```python
from build123d import *

# Parameters (mm, degrees)
SKETCH1_W                                        = 435
SKETCH1_H                                        = 385
BOSS_EXTRUDE1_DEPTH                              = 4
FILLET1_R                                        = 20
SKETCH2_R                                        = 1.555451355
SKETCH2_R_2                                      = 1.5
SKETCH2_R_3                                      = 1.924870622
CUT_EXTRUDE1_DEPTH                               = 10
CUT_EXTRUDE2_DEPTH                               = 4
HOLE_SIZE_BY_HEXALOBULAR_COUNTERSUNK_D           = 6.6
HOLE_SIZE_BY_HEXALOBULAR_COUNTERSUNK_DEPTH       = 7.5
HOLE_SIZE_BY_HEXALOBULAR_COUNTERSUNK_CSINK_D     = 12.8
HOLE_SIZE_BY_HEXALOBULAR_COUNTERSUNK_CSINK_ANGLE = 90
HOLE_SIZE_BY_HEXALOBULAR_COUNTERSUNK_TIP         = 1.982840043
SKETCH6_R                                        = 17.5
CUT_EXTRUDE3_DEPTH                               = 4
SKETCH7_R                                        = 1.6
CUT_EXTRUDE4_DEPTH                               = 4


with BuildPart() as part:
    # Sketch1 → Boss-Extrude1 (new body)
    with BuildSketch(Plane(origin=(0, 0, 0), x_dir=(1, 0, 0), z_dir=(0, 1, 0))):
        Rectangle(SKETCH1_W, SKETCH1_H)
    extrude(amount=BOSS_EXTRUDE1_DEPTH)

    # Fillet1
    fillet1_edges = [part.edges().sort_by_distance(p)[0] for p in [
        (217.5, 2, 192.5),
        (-217.5, 2, 192.5),
        (-217.5, 2, -192.5),
        (217.5, 2, -192.5),
    ]]
    fillet(fillet1_edges, radius=FILLET1_R)

    # Sketch2 → Cut-Extrude1 (cut)
    with BuildSketch(Plane(origin=(0, 4, 0), x_dir=(1, 0, 0), z_dir=(0, 1, 0))):
        with Locations(Location((-42.5, 0, 0), (0, 0, 270))):
            Circle(SKETCH2_R)
        with Locations(Location((-55.5, 7.5, 0), (0, 0, 270))):
            Circle(SKETCH2_R_2)
        with Locations(Location((-55.5, -7.5, 0), (0, 0, 270))):
            Circle(SKETCH2_R_3)
    extrude(amount=-CUT_EXTRUDE1_DEPTH, mode=Mode.SUBTRACT)

    # Sketch3 → Cut-Extrude2 (cut)
    with BuildSketch(Plane(origin=(0, 4, 0), x_dir=(1, 0, 0), z_dir=(0, 1, 0))):
        with BuildLine():
            Line((-24.5, -25), (69.5, -25))
            ThreePointArc((69.5, -25), (71.621320344, -24.121320344), (72.5, -22))
            Line((72.5, -22), (72.5, 22))
            ThreePointArc((72.5, 22), (71.621320344, 24.121320344), (69.5, 25))
            Line((69.5, 25), (-24.5, 25))
            ThreePointArc((-24.5, 25), (-26.621320344, 24.121320344), (-27.5, 22))
            Line((-27.5, 22), (-27.5, -22))
            ThreePointArc((-27.5, -22), (-26.621320344, -24.121320344), (-24.5, -25))
        make_face()
    extrude(amount=-CUT_EXTRUDE2_DEPTH, mode=Mode.SUBTRACT)

    # Hole Size (% by) Hexalobular Countersunk Head Screw Type1
    with Locations(Plane(origin=(0, 4, 0), x_dir=(1, 0, 0), z_dir=(0, 1, 0))):
        with Locations((-55.5, -7.5), (-42.5, 0), (-55.5, 7.5)):
            CounterSinkHole(HOLE_SIZE_BY_HEXALOBULAR_COUNTERSUNK_D / 2, HOLE_SIZE_BY_HEXALOBULAR_COUNTERSUNK_CSINK_D / 2, depth=HOLE_SIZE_BY_HEXALOBULAR_COUNTERSUNK_DEPTH, counter_sink_angle=HOLE_SIZE_BY_HEXALOBULAR_COUNTERSUNK_CSINK_ANGLE)
            with Locations((0, 0, -(HOLE_SIZE_BY_HEXALOBULAR_COUNTERSUNK_DEPTH + HOLE_SIZE_BY_HEXALOBULAR_COUNTERSUNK_TIP / 2))):  # 118° drill point
                Cone(0, HOLE_SIZE_BY_HEXALOBULAR_COUNTERSUNK_D / 2, HOLE_SIZE_BY_HEXALOBULAR_COUNTERSUNK_TIP, mode=Mode.SUBTRACT)

    # Sketch6 → Cut-Extrude3 (cut)
    with BuildSketch(Plane.XZ):
        with Locations(Location((-48, 100, 0), (0, 0, 270))):
            Circle(SKETCH6_R)
        with Locations(Location((97, 100, 0), (0, 0, 270))):
            Circle(SKETCH6_R)
        with Locations(Location((-48, -100, 0), (0, 0, 270))):
            Circle(SKETCH6_R)
        with Locations(Location((97, -100, 0), (0, 0, 270))):
            Circle(SKETCH6_R)
    extrude(amount=-CUT_EXTRUDE3_DEPTH, mode=Mode.SUBTRACT)

    # Sketch7 → Cut-Extrude4 (cut)
    with BuildSketch(Plane.XZ):
        with Locations(Location((-190, 175, 0), (0, 0, 270))):
            Circle(SKETCH7_R)
        with Locations(Location((-190, 0, 0), (0, 0, 270))):
            Circle(SKETCH7_R)
        with Locations(Location((-190, -175, 0), (0, 0, 270))):
            Circle(SKETCH7_R)
        with Locations(Location((190, 175, 0), (0, 0, 270))):
            Circle(SKETCH7_R)
        with Locations(Location((190, 0, 0), (0, 0, 270))):
            Circle(SKETCH7_R)
        with Locations(Location((190, -175, 0), (0, 0, 270))):
            Circle(SKETCH7_R)
    extrude(amount=-CUT_EXTRUDE4_DEPTH, mode=Mode.SUBTRACT)


solid = part.part
```
For this review, take the finished solid that the model builds, in its own axes (mm). Coordinates: 2 decimals unless noted, no trailing zeros. Loops run counter-clockwise (first coordinate to the right, second up) from the corner with the lowest first, then second, coordinate; pieces in that order, holes last. Notation, with made-up numbers: (-24, 65.5) -> (3, 65.5) arc R20 ccw to (3, 93.5) -> close; hole circle Ø10 at (44.5, -22). An arc over 180 degrees is marked (long way). Return JSON: item names as keys, results as strings. Group by question number.
(1) Mouldability with a two-part tool opening along Z and no side actions: class faces 1 (the flat face through (-3, 0, 40)), 2 (the cylindrical face through (-211.797, 2.028, -186.486)), 3 (the cylindrical face through (211.486, 2.028, 186.797)), 4 (the cylindrical face through (108.827, 1.972, 112.898)) as pulls with the +Z half, pulls with the -Z half, needs draft (parallel to the pull), parting line crosses it, or undercut.
(2) Consider section A-A, the plane z = 100. Give the boundary of the cut face in (x, y), plus the area to 3 significant figures.
(3) Consider section C-C, the plane x = 97. Give the boundary of the cut face in (y, z), plus the area to 3 significant figures.
(4) Consider section B-B, the plane y = 2.6. Count the separate pieces of the cut face and the enclosed holes in it, plus the area to 3 significant figures.
(5) For pin 1 Ø3.5 at (x, z) = (190, 175) entering from -Y; pin 2 Ø7.5 at (x, z) = (-42.5, 0) entering from +Y, all flat-tipped, find the tip position at first contact; note any pin that passes through.
(6) To check wall thickness, follow L1, parallel to Z at x = 97.5, y = 0.25; L2, parallel to X at y = 1.9, z = -100; L3, parallel to Z at x = 190, y = 1.6. State the ranges of each line that lie inside material, in increasing order.
Results below:
{
 "1": {"face 1": "needs draft", "face 2": "pulls with the -Z half", "face 3": "pulls with the +Z half", "face 4": "undercut"},
 "2": {"outline": "(-217.5, 0) -> (-65.5, 0) -> (-65.5, 4) -> (-217.5, 4) -> close; (-30.5, 0) -> (79.5, 0) -> (79.5, 4) -> (-30.5, 4) -> close; (114.5, 0) -> (217.5, 0) -> (217.5, 4) -> (114.5, 4) -> close", "area": "1,460 mm2"},
 "3": {"outline": "(0, -192.5) -> (4, -192.5) -> (4, -117.5) -> (0, -117.5) -> close; (0, -82.5) -> (4, -82.5) -> (4, 82.5) -> (0, 82.5) -> close; (0, 117.5) -> (4, 117.5) -> (4, 192.5) -> (0, 192.5) -> close", "area": "1,260 mm2"},
 "4": {"separate pieces": "1", "enclosed holes": "14", "area": "158,000 mm2"},
 "5": {"pin 1": "stops at y = 0", "pin 2": "stops at y = 1.35"},
 "6": {"L1": "z = -192.5 to -117.49, -82.51 to 82.51, 117.49 to 192.5", "L2": "x = -217.5 to -65.5, -30.5 to 79.5, 114.5 to 217.5", "L3": "z = -192.5 to -176.6, -173.4 to -1.6, 1.6 to 173.4, 176.6 to 192.5"}
}
